Drawing for the job (mm, zero at the part's lowest x, y, z). A direction names the side the tool comes from. Give positions to 0.01 mm unless a question says otherwise; leave off trailing zeros. Order: outer loops, then holes, each group sorted by start corner. A loop starts at its lowest first (then second) coordinate and runs counter-clockwise, first axis right, second up. Notation, with made-up numbers: M -9.5,-36.5 L 36.5,-36.5 A22 cw 36.5,-28.5 Z; hole C -9.75,50.25 d6. An arc over 180 degrees is marked long. Answer as a JSON object with one key per item and string values.
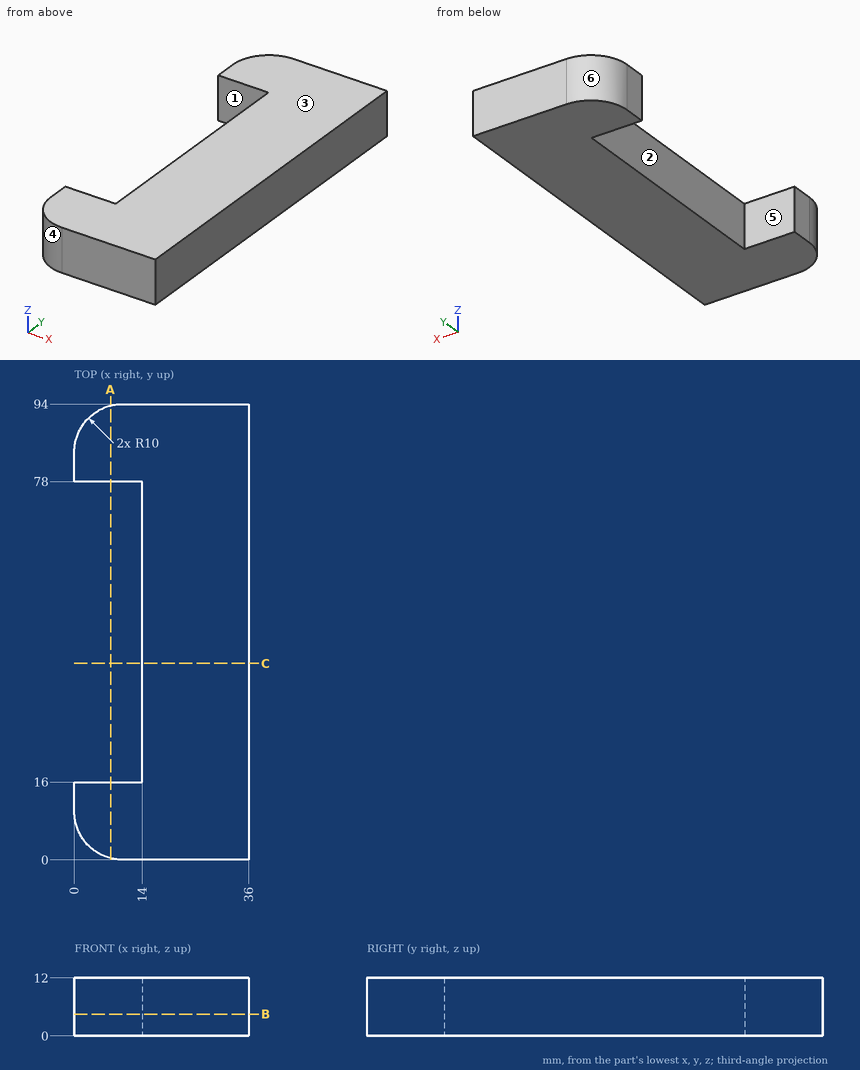
1. Which spindle directions (+Z, -Z, +X, -X, +Y, -Y) get a long thin tool onto all of the face, cutting with end or side? Do the marked faces 5 and 6. Say none if no direction does.
Worked answers:
{"face 5": "+Z, -Z, -X", "face 6": "+Z, -Z, -X, +Y"}
2. Probe line 1 along X through (y, z) = (35.5, 4); line 2 along Y through (x, z) = (3.5, 10); line 3 along Y through (x, z) = (2.5, 3.75). List the from-to ranges inside material, lowest first.
Worked answers:
{"line 1": "x = 14 to 36", "line 2": "y = 2.4 to 16, 78 to 91.6", "line 3": "y = 3.39 to 16, 78 to 90.61"}
3. Cut at C-C on y = 40.5. Give the cut face in (x, z).
Worked answers:
{"outline": "M 14,0 L 36,0 L 36,12 L 14,12 Z"}
4. Two-plate mould, pull along Y, no slides. Class the marked faces 1, 2, 3 and 4: +Y half, -Y half, draft (parallel to the pull), parting line (faces both ways), or undercut.
Worked answers:
{"face 1": "undercut", "face 2": "undercut", "face 3": "draft", "face 4": "-Y half"}
5. Pin check, flat tip, straight feed: P1, Ø5, axis at y = 36.5, z = 10, coming from the -X side. Stop position of the tip, or through.
Worked answers:
{"P1": "stops at x = 14"}
6. Cut at A-A on x = 7.5. Give the cut face in (y, z).
Worked answers:
{"outline": "M 0.32,0 L 16,0 L 16,12 L 0.32,12 Z; M 78,0 L 93.68,0 L 93.68,12 L 78,12 Z"}
7. Cut at B-B on z = 4.5. Give the cut face in (x, y), plus the area to 3 significant figures.
Worked answers:
{"outline": "M 0,10 A10 ccw 10,0 L 36,0 L 36,94 L 10,94 A10 ccw 0,84 L 0,78 L 14,78 L 14,16 L 0,16 Z", "area": "2,470 mm^2"}
